Work out the finished part from the listing and answer in its coordinate system (mm). Face numbers are marked on the shaded views. A direction names the side the tool comes from. Round coordinates to 2 decimals unless told otherwise and drop trailing zeros. Order: outer loops, then holes, each group sorted by start corner. A loop starts at its lowest first (then second) coordinate and runs counter-clockwise, first axis right, second up. Notation, with made-up numbers: (-23.75, 3) -> (26.25, 3) arc R22 cw to (26.25, 42) -> close; hole circle Ø6 at (88, 43.5). An arc over 180 degrees is marked (long way). Use one line per item in the form item = value.
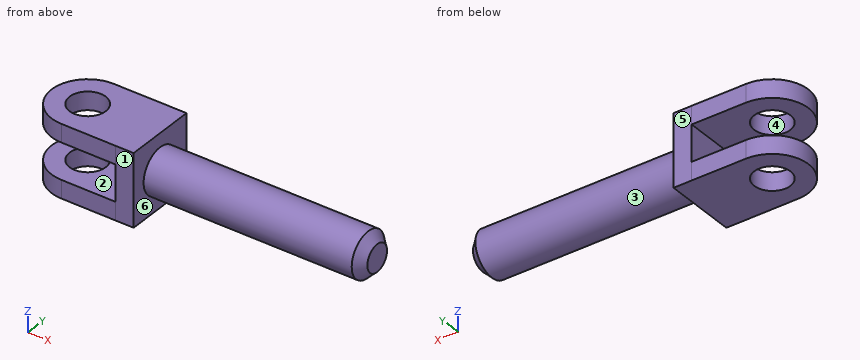
```python
from build123d import *

# Parameters (mm, degrees)
CLEVIS_BLOCK_SKETCH_W  = 3.175
CLEVIS_BLOCK_SKETCH_H  = 12.7
CLEVIS_BLOCK_DEPTH     = 6.35
SHANK_SKETCH_7_95_R    = 3.95
SHANK_7_95_DEPTH       = 38.1
SHANK_END_CHAMFER_SIZE = 1.5875
CLEVIS_EAR_SKETCH_R    = 3.175
CLEVIS_EAR_DEPTH       = 3.175


with BuildPart() as part:
    # Clevis Block Sketch → Clevis Block (new, symmetric)
    with BuildSketch(Plane.XY):
        with Locations((1.5875, 0)):
            Rectangle(CLEVIS_BLOCK_SKETCH_W, CLEVIS_BLOCK_SKETCH_H)
    extrude(amount=CLEVIS_BLOCK_DEPTH, both=True)

    # Shank Sketch Ø7.95 → Shank Ø7.95 (add)
    with BuildSketch(Plane(origin=(3.175, 0, 0), x_dir=(0, 0, -1), z_dir=(1, 0, 0))):
        with Locations(Location((0, 0, 0), (0, 0, 270))):
            Circle(SHANK_SKETCH_7_95_R)
    extrude(amount=SHANK_7_95_DEPTH)

    # Shank End Chamfer
    shank_end_chamfer_edges = [part.edges().sort_by_distance(p)[0] for p in [
        (41.275, 3.95, 0),
    ]]
    chamfer(shank_end_chamfer_edges, length=SHANK_END_CHAMFER_SIZE)

    # Clevis Ear Sketch → Clevis Ear (add)
    with BuildSketch(Plane(origin=(0, 0, -6.35), x_dir=(-1, 0, 0), z_dir=(0, 0, -1))):
        with BuildLine():
            Line((9.525, 6.332334812), (0, 6.35))
            Line((0, 6.35), (0, -6.35))
            Line((0, -6.35), (9.525, -6.332334812))
            ThreePointArc((9.525, -6.332334812), (15.857334812, 0), (9.525, 6.332334812))
        make_face()
        with Locations((9.525, 0)):
            Circle(CLEVIS_EAR_SKETCH_R, mode=Mode.SUBTRACT)
    clevis_ear = extrude(amount=-CLEVIS_EAR_DEPTH)

    # Clevis Ear Mirror: Clevis Ear across plane
    add(clevis_ear.mirror(Plane.XY))


solid = part.part
```
Item 1: The part is cut by section D-D, the plane x = -8. Give the vertices of the cut face in (y, z) (3 decimals), and give its area (3 significant figures).
Findings:
outline = (-6.335, -6.35) -> (-2.785, -6.35) -> (-2.785, -3.175) -> (-6.335, -3.175) -> close; (-6.335, 3.175) -> (-2.785, 3.175) -> (-2.785, 6.35) -> (-6.335, 6.35) -> close; (2.785, -6.35) -> (6.335, -6.35) -> (6.335, -3.175) -> (2.785, -3.175) -> close; (2.785, 3.175) -> (6.335, 3.175) -> (6.335, 6.35) -> (2.785, 6.35) -> close
area = 45.1 mm^2
Item 2: Consider line 1 along Z through (x, y) = (-3, 1.5) (3 decimals); line 2 along Z through (x, y) = (25, 0); line 3 along X through (y, z) = (2, 4.75) (3 decimals). Determine where each line is inside the solid, lowest interval first.
Findings:
line_1 = -6.35 to -3.175, 3.175 to 6.35
line_2 = -3.95 to 3.95
line_3 = -15.533 to -11.991, -7.059 to 3.175
Item 3: Determine the mould class of the marked faces 4, 5 and 6 for opening direction Y: released by +Y, released by -Y, zero draft, split by the parting line, or undercut.
Findings:
face_4 = undercut
face_5 = released by +Y
face_6 = zero draft
Item 4: Flat-ended cylindrical pins translate along their axes: P1, Ø2, axis at x = 33, y = 2, coming from the -Z side; P2, Ø3, axis at y = 3.5, z = 4.5, coming from the -X side; P3, Ø3, axis at x = 26, y = 0.5, coming from the -Z side. Find the tip coordinate at first contact, or state that the pin passes through.
Findings:
P1 = -3.82
P2 = -15.53
P3 = -3.95
Item 5: For the marked faces 1, 2 and 3, determine the directions among +Z, -Z, +X, -X, +Y, -Y from which every point of the face is accessible in a straight line to the end or side of a thin tool.
Findings:
face_1 = +Z, -Z, +X, -X, -Y
face_2 = -X, +Y, -Y
face_3 = +X
Item 6: The part is cut by section C-C, the plane x = -1.5. Give the vertices of the cut face in (y, z) (3 decimals).
Findings:
outline = (-6.347, -6.35) -> (6.347, -6.35) -> (6.347, -3.175) -> (-6.347, -3.175) -> close; (-6.347, 3.175) -> (6.347, 3.175) -> (6.347, 6.35) -> (-6.347, 6.35) -> close
Item 7: The part is cut by section A-A, the plane y = 0. Give the number of separate pieces and of enclosed holes in the cut face, and give its area (3 significant figures).
Findings:
separate_pieces = 3
enclosed_holes = 0
area = 399 mm^2
